from build123d import *

# Parameters (mm, degrees)
SKETCH1_R           = 15
BOSS_EXTRUDE1_DEPTH = 15
SKETCH6_R           = 4.1
CUT_EXTRUDE3_DEPTH  = 50
SKETCH8_R           = 8.75
CUT_EXTRUDE5_DEPTH  = 6
CHAMFER2_SIZE       = 0.5
CHAMFER3_SIZE       = 0.5


with BuildPart() as part:
    # Sketch1 → Boss-Extrude1 (new body)
    with BuildSketch(Plane.XY):
        Circle(SKETCH1_R)
    extrude(amount=BOSS_EXTRUDE1_DEPTH)

    # Sketch6 → Cut-Extrude3 (cut)
    with BuildSketch(Plane(origin=(0, 0, 0), x_dir=(-1, 0, 0), z_dir=(0, 0, -1))):
        Circle(SKETCH6_R)
    extrude(amount=-CUT_EXTRUDE3_DEPTH, mode=Mode.SUBTRACT)

    # Sketch8 → Cut-Extrude5 (cut)
    with BuildSketch(Plane.XY.offset(15)):
        Circle(SKETCH8_R)
    extrude(amount=-CUT_EXTRUDE5_DEPTH, mode=Mode.SUBTRACT)

    # Chamfer2
    chamfer2_edges = [part.edges().sort_by_distance(p)[0] for p in [
        (-8.75, 0, 15),
    ]]
    chamfer(chamfer2_edges, length=CHAMFER2_SIZE)

    # Chamfer3
    chamfer3_edges = [part.edges().sort_by_distance(p)[0] for p in [
        (-15, 0, 0),
        (-15, 0, 15),
        (4.1, 0, 0),
    ]]
    chamfer(chamfer3_edges, length=CHAMFER3_SIZE)


solid = part.part
Could you check a few things on this model? Use its own coordinates, in mm. A direction names the side the tool comes from. Give positions to 0.01 mm unless a question says otherwise; leave off trailing zeros. Order: outer loops, then holes, each group sorted by start corner. A loop starts at its lowest first (then second) coordinate and runs counter-clockwise, first axis right, second up.
Item 1: If we mould it in two halves opening along Y, with no side actions, what happens to faces 3 (the face through (-3.4, 3.4, 0)), 4 (the face through (-14.985, 0.66, 7.402)), 5 (the face through (-6.944, -5.324, 11.788))? For each: pulls with the +Y half, pulls with the -Y half, needs draft (parallel to the pull), parting line crosses it, or undercut.
Item 2: If we section it at C-C, the plane z = 3.75: Write out the boundary of the cut face in (x, y).
Item 3: For faces 1 (the face through (4, -2, 9)), 2 (the face through (-0.2, -9.5, 15)), which set-ups out of +Z, -Z, +X, -X, +Y, -Y let a thin tool reach every point of the face, with its end or its side?
Item 4: I need wall thicknesses on line 1 (Y direction, x = 0, z = 5); line 2 (Y direction, x = 0, z = 10.85); line 3 (X direction, y = -1, z = 3.5). Which ranges of each line are inside material? Lowest first, please.
Item 5: I'm going to push flat-ended pins straight in: pin 1 (1 mm diameter, centred on x = -1, y = -2.5, fed in from -Z); pin 2 (2 mm diameter, centred on y = 11, z = 2, fed in from +X); pin 3 (2 mm diameter, centred on y = -4, z = 5, fed in from -X); pin 4 (3 mm diameter, centred on x = -6, z = 6, fed in from +Y). Where does each tip first touch, or does it pass through?
Item 6: If we section it at A-A, the plane y = 0: Write out the boundary of the cut face in (x, z).
Values:
1. face 3: needs draft
1. face 4: parting line crosses it
1. face 5: undercut
2. outline: circle Ø30 at (0, 0); hole circle Ø8.2 at (0, 0)
3. face 1: +Z
3. face 2: +Z, +X, -X, +Y, -Y
4. line 1: y = -15 to -4.1, 4.1 to 15
4. line 2: y = -15 to -8.75, 8.75 to 15
4. line 3: x = -14.97 to -3.98, 3.98 to 14.97
5. pin 1: passes through
5. pin 2: stops at x = 11.18
5. pin 3: stops at x = -14.7
5. pin 4: stops at y = 14.31
6. outline: (-15, 0.5) - (-14.5, 0) - (-4.6, 0) - (-4.1, 0.5) - (-4.1, 9) - (-8.75, 9) - (-8.75, 14.5) - (-9.25, 15) - (-14.5, 15) - (-15, 14.5) - close; (4.1, 0.5) - (4.6, 0) - (14.5, 0) - (15, 0.5) - (15, 14.5) - (14.5, 15) - (9.25, 15) - (8.75, 14.5) - (8.75, 9) - (4.1, 9) - close
